Could you check a few things on this model? Use its own coordinates, in mm. Face numbers are marked on the shaded views. A direction names the side the tool comes from. Coordinates: 2 decimals unless noted, no trailing zeros. Order: outer loops, then holes, each group sorted by start corner. A loop starts at its lowest first (then second) coordinate and runs counter-clockwise, first axis right, second up. Notation, with made-up numbers: (3, 51.25) - (40, 51.25) arc R26 ccw to (40, 76.25) - close; hole circle Ø9 at (-9, -39.5). An arc over 180 degrees is marked (long way). Answer as a JSON object with one key per item and string values. Group by question number.
(1) Imagine slicing it at A-A, the plane z = -4.75. Write out the boundary of the cut face in (x, y), and give its area (3 significant figures).
(2) Please list where these lines run through material, in increasing order: probe 1 along X at (y, z) = (9, 0); probe 2 along Y at (x, z) = (10, 0); probe 3 along Z at (x, y) = (22.5, 5.75).
(3) Will these pins go through, and if not, where does the flat tip stop? P1, Ø1.5, axis at x = 61, z = -4, coming from the -Y side; P2, Ø7.5, axis at y = 101.5, z = 0.5, coming from the +X side; P3, Ø4, axis at y = 120, z = 0, coming from the -X side; P4, Ø4.5, axis at x = 115.5, z = 0, coming from the +Y side.
(4) Imagine slicing it at B-B, the plane x = 128. Write out the boundary of the cut face in (y, z).
(5) Which directions (+Z, -Z, +X, -X, +Y, -Y) give clear straight access to the entire face, cutting with the end or side of a thin tool? Please do the marked faces 1 and 2.
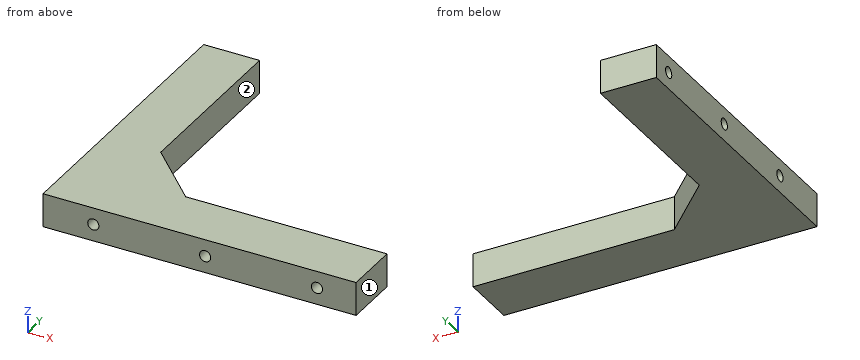
from build123d import *

# Parameters (mm, degrees)
EXTRUDE_1_DEPTH                  = 7.5
HOLE_WIZARD_M6_1_D               = 5
HOLE_WIZARD_M6_1_DEPTH           = 12.5
HOLE_WIZARD_M6_1_TIP             = 1.502151548
HOLE_WIZARD_M6_1_ON_FACE_2_D     = 5
HOLE_WIZARD_M6_1_ON_FACE_2_DEPTH = 12.5
HOLE_WIZARD_M6_1_ON_FACE_2_TIP   = 1.502151548


with BuildPart() as part:
    # 草图1 → 凸台-拉伸1 (new, symmetric)
    with BuildSketch(Plane.XY):
        Polygon((0, 130), (0, 0), (140, 0), (140, 25), (50, 25), (25, 50), (25, 130), align=None)
    extrude(amount=EXTRUDE_1_DEPTH, both=True)

    # M6 螺纹孔1
    with Locations(Plane(origin=(122.5, 0, 0), x_dir=(0, 0, -1), z_dir=(0, -1, 0))):
        with Locations((0, 0), (0, -50), (0, -100)):
            Hole(HOLE_WIZARD_M6_1_D / 2, depth=HOLE_WIZARD_M6_1_DEPTH)
            with Locations((0, 0, -(HOLE_WIZARD_M6_1_DEPTH + HOLE_WIZARD_M6_1_TIP / 2))):  # 118° drill point
                Cone(0, HOLE_WIZARD_M6_1_D / 2, HOLE_WIZARD_M6_1_TIP, mode=Mode.SUBTRACT)

    # M6 螺纹孔1 on face 2
    with Locations(Plane(origin=(0, 30, 0), x_dir=(0, 0, -1), z_dir=(-1, 0, 0))):
        with Locations((0, 0), (0, -45), (0, -90)):
            Hole(HOLE_WIZARD_M6_1_ON_FACE_2_D / 2, depth=HOLE_WIZARD_M6_1_ON_FACE_2_DEPTH)
            with Locations((0, 0, -(HOLE_WIZARD_M6_1_ON_FACE_2_DEPTH + HOLE_WIZARD_M6_1_ON_FACE_2_TIP / 2))):  # 118° drill point
                Cone(0, HOLE_WIZARD_M6_1_ON_FACE_2_D / 2, HOLE_WIZARD_M6_1_ON_FACE_2_TIP, mode=Mode.SUBTRACT)


solid = part.part
Result set:
{
 "1": {"outline": "(0, 0) - (140, 0) - (140, 25) - (50, 25) - (25, 50) - (25, 130) - (0, 130) - close", "area": "6,440 mm^2"},
 "2": {"probe 1": "x = 0 to 20, 25 to 70, 75 to 120, 125 to 140", "probe 2": "y = 0 to 27.5, 32.5 to 72.5, 77.5 to 117.5, 122.5 to 130", "probe 3": "z = -7.5 to -2.5, 2.5 to 7.5"},
 "3": {"P1": "stops at y = 0", "P2": "stops at x = 25", "P3": "stops at x = 12.8", "P4": "stops at y = 25"},
 "4": {"outline": "(0, -7.5) - (25, -7.5) - (25, 7.5) - (0, 7.5) - close"},
 "5": {"face 1": "+Z, -Z, +X, +Y, -Y", "face 2": "+Z, -Z, +X, +Y"}
}
